```python
from build123d import *

# Parameters (mm, degrees)
SKETCH1_R           = 6.5
BOSS_EXTRUDE1_DEPTH = 15
CUT_EXTRUDE1_START  = -13
SKETCH2_R           = 13
CUT_EXTRUDE1_DEPTH  = 2
FILLET1_R           = 15
SKETCH4_R           = 27.5
BOSS_EXTRUDE2_DEPTH = 2
SKETCH5_R           = 7.25
CUT_EXTRUDE2_DEPTH  = 30
SKETCH6_R           = 35
CUT_EXTRUDE3_DEPTH  = 50
FILLET2_R           = 15


with BuildPart() as part:
    # Sketch1 → Boss-Extrude1 (new body)
    with BuildSketch(Plane.XY):
        with BuildLine():
            ThreePointArc((30.608172596, 51.605617624), (0.11519166, 59.999889424), (-30.409796101, 51.722763858))
            ThreePointArc((-30.409796101, 51.722763858), (-50.011440089, 50.39698265), (-51.487710544, 30.806097821))
            ThreePointArc((-51.487710544, 30.806097821), (-59.999557696, 0.230382895), (-51.722763858, -30.409796101))
            ThreePointArc((-51.722763858, -30.409796101), (-50.39698265, -50.011440089), (-30.806097821, -51.487710544))
            ThreePointArc((-30.806097821, -51.487710544), (-0.230382895, -59.999557696), (30.409796101, -51.722763858))
            ThreePointArc((30.409796101, -51.722763858), (50.011440089, -50.39698265), (51.487710544, -30.806097821))
            ThreePointArc((51.487710544, -30.806097821), (59.999889424, -0.11519166), (51.605617624, 30.608172596))
            ThreePointArc((51.605617624, 30.608172596), (50.204581464, 50.204581464), (30.608172596, 51.605617624))
        make_face()
        with Locations((39.597979746, 39.597979746)):
            Circle(SKETCH1_R, mode=Mode.SUBTRACT)
        with Locations((-39.445642887, 39.749732794)):
            Circle(SKETCH1_R, mode=Mode.SUBTRACT)
        with Locations((-39.749732794, -39.445642887)):
            Circle(SKETCH1_R, mode=Mode.SUBTRACT)
        with Locations((39.445642887, -39.749732794)):
            Circle(SKETCH1_R, mode=Mode.SUBTRACT)
    extrude(amount=BOSS_EXTRUDE1_DEPTH)

    # Sketch2 → Cut-Extrude1 (cut)
    with BuildSketch(Plane.XY.offset(15).offset(CUT_EXTRUDE1_START)):
        with Locations((-39.445642887, 39.749732794)):
            Circle(SKETCH2_R)
        with Locations((39.597979746, 39.597979746)):
            Circle(SKETCH2_R)
        with Locations((39.445642887, -39.749732794)):
            Circle(SKETCH2_R)
        with Locations((-39.749732794, -39.445642887)):
            Circle(SKETCH2_R)
    extrude(amount=-CUT_EXTRUDE1_DEPTH, mode=Mode.SUBTRACT)

    # Sketch3 → Revolve1 (revolve)
    with BuildSketch(Plane(origin=(0, 0, 0), x_dir=(1, 0, 0), z_dir=(0, 1, 0))):
        Polygon((-42.5, 0), (-42.5, 43), (-17.5, 43), (-17.5, 50), (-15, 50), (-15, 55), (-17.5, 55), (-17.5, 60), (0, 60), (0, 0), align=None)
    revolve(axis=Axis((0, 0, -60), (0, 0, 1)))

    # Fillet1
    fillet1_edges = [part.edges().sort_by_distance(p)[0] for p in [
        (42.5, 0, -43),
    ]]
    fillet(fillet1_edges, radius=FILLET1_R)

    # Sketch4 → Boss-Extrude2 (add)
    with BuildSketch(Plane(origin=(0, 0, -43), x_dir=(-1, 0, 0), z_dir=(0, 0, -1))):
        Circle(SKETCH4_R)
    extrude(amount=BOSS_EXTRUDE2_DEPTH)

    # Sketch5 → Cut-Extrude2 (cut)
    with BuildSketch(Plane(origin=(0, 0, -60), x_dir=(-1, 0, 0), z_dir=(0, 0, -1))):
        Circle(SKETCH5_R)
    extrude(amount=-CUT_EXTRUDE2_DEPTH, mode=Mode.SUBTRACT)

    # Sketch6 → Cut-Extrude3 (cut)
    with BuildSketch(Plane.XY.offset(15)):
        Circle(SKETCH6_R)
    extrude(amount=-CUT_EXTRUDE3_DEPTH, mode=Mode.SUBTRACT)

    # Fillet2
    fillet2_edges = [part.edges().sort_by_distance(p)[0] for p in [
        (-35, 0, -35),
    ]]
    fillet(fillet2_edges, radius=FILLET2_R)


solid = part.part
```
Source: CAD feature listing. Evaluate the final solid. Frame: model axes, mm. A direction names the side the tool comes from. Give positions to 0.01 mm unless a question says otherwise; leave off trailing zeros. Loops run counter-clockwise (first coordinate to the right, second up) from the corner with the lowest first, then second, coordinate; pieces in that order, holes last. Notation, with made-up numbers: (-30, 31.25) -> (-17, 31.25) arc R18 ccw to (-17, 37.25) -> close; hole circle Ø5 at (76.25, 64.5). An arc over 180 degrees is marked (long way). Use a Markdown table: item, result. Add a question column.
(1) Section query D-D (z = -48). Output: boundary loops of the cut face in (x, y).
(2) First-contact query: pin 1 Ø13 at (x, y) = (34, 42) entering from -Z; pin 2 Ø2 at (y, z) = (1, -3.5) entering from -X; pin 3 Ø10 at (y, z) = (-6, -19.5) entering from +X; pin 4 Ø8 at (y, z) = (39, -45) entering from -X. Flat tips, straight axial feed; report the tip coordinate or a pass-through.
(3) Access query for faces 5 (the face through (50.415, 49.99, 7.395)), 6 (the face through (13, -8, -55)), 7 (the face through (-28, -21, -2)), 8 (the face through (-33.75, -50.98, 1.01)). Directions: +Z, -Z, +X, -X, +Y, -Y. A direction counts if a zero-diameter tool reaches every point of the face in a straight line with its end or side. Return the directions, or none.
(4) Section query C-C (x = -44). Output: boundary loops of the cut face in (y, z), then the cut area to 3 significant figures.
(5) Pull-direction query (Y, two-part tool) for faces 1 (the face through (-13, -8, -50)), 2 (the face through (0.563, 59.997, 7.395)), 3 (the face through (-37, 46, 2)), 4 (the face through (49.8, -50.6, 7.4)); classes: +Y half, -Y half, draft (parallel to the pull), parting line (faces both ways), or undercut.
(6) Ray query, line 1 (Z direction, x = -4, y = 45.5); line 2 (Z direction, x = 19.5, y = 7); line 3 (Y direction, x = -9, z = -13). Return the intervals inside material, ascending.
Checked values:
| question | item | result |
|---|---|---|
| 1 | outline | circle Ø35 at (0, 0); hole circle Ø14.5 at (0, 0) |
| 2 | pin 1 | z = 2 |
| 2 | pin 2 | x = -42.5 |
| 2 | pin 3 | x = 42.49 |
| 2 | pin 4 | through |
| 3 | face 5 | +Z, -Z |
| 3 | face 6 | none |
| 3 | face 7 | +Z |
| 3 | face 8 | -Z |
| 4 | outline | (-53.83, 0) -> (-51.73, 0) -> (-51.73, 2) -> (-44.36, 2) -> (-44.36, 15) -> (-53.83, 15) -> close; (-34.53, 2) -> (-27.16, 2) -> (-27.16, 0) -> (27.57, 0) -> (27.57, 2) -> (35.11, 2) -> (35.11, 15) -> (-34.53, 15) -> close; (44.39, 2) -> (51.93, 2) -> (51.93, 0) -> (54.04, 0) -> (54.04, 15) -> (44.39, 15) -> close |
| 4 | area | 1,270 mm^2 |
| 5 | face 1 | draft |
| 5 | face 2 | +Y half |
| 5 | face 3 | undercut |
| 5 | face 4 | undercut |
| 6 | line 1 | 0 to 15 |
| 6 | line 2 | -45 to -34.98 |
| 6 | line 3 | -41.54 to -33.82, 33.82 to 41.54 |
